Check sheet for the modelled part. Datum: model origin and axes. Units: mm. Face numbers are marked on the shaded views. Round coordinates to 2 decimals unless told otherwise and drop trailing zeros. Order: outer loops, then holes, each group sorted by start corner. A loop starts at its lowest first (then second) coordinate and runs counter-clockwise, first axis right, second up. Notation, with made-up numbers: (45.5, 57.5) -> (92.5, 57.5) arc R17 ccw to (92.5, 85.5) -> close; hole circle Ø7 at (87, 39.5). An arc over 180 degrees is marked (long way). Answer in a Markdown table with one row per item. Add a question column.
1. Sectioned sample at B-B, the plane y = -7.5. Record the boundary of the cut face in (x, z), then the cut area to 3 significant figures.
2. Sectioned sample at A-A, the plane z = 10.5. Record the boundary of the cut face in (x, y).
3. Sectioned sample at C-C, the plane x = 5.75. Record the boundary of the cut face in (y, z), then the cut area to 3 significant figures.
4. Draft check along X on the marked faces 1, 2, 3 and 4. Enter one of: +X half, -X half, draft (parallel to the pull), parting line (faces both ways), or undercut.
5. Material ranges on L1, parallel to Y at x = 0, z = 13; L2, parallel to X at y = 3.03, z = 10; L3, parallel to X at y = 2, z = 2, recorded low to high. Write a range as from..to.
```python
from build123d import *

# Parameters (mm, degrees)
SKETCH1_W             = 15
SKETCH1_H             = 20
BOSS_EXTRUDE1_DEPTH   = 17.5
CHAMFER1_SIZE         = 3
M6_TAPPED_HOLE1_D     = 5
M6_TAPPED_HOLE1_DEPTH = 15
M6_TAPPED_HOLE1_TIP   = 1.502151548


with BuildPart() as part:
    # Sketch1 → Boss-Extrude1 (new, symmetric)
    with BuildSketch(Plane.XY):
        Rectangle(SKETCH1_W, SKETCH1_H)
    extrude(amount=BOSS_EXTRUDE1_DEPTH, both=True)

    # Chamfer1
    chamfer1_edges = [part.edges().sort_by_distance(p)[0] for p in [
        (7.5, -10, 0),
        (-7.5, -10, 0),
    ]]
    chamfer(chamfer1_edges, length=CHAMFER1_SIZE)

    # M6 Tapped Hole1
    with Locations(Plane.XY.offset(17.5)):
        with Locations((0, 3.03)):
            Hole(M6_TAPPED_HOLE1_D / 2, depth=M6_TAPPED_HOLE1_DEPTH)
            with Locations((0, 0, -(M6_TAPPED_HOLE1_DEPTH + M6_TAPPED_HOLE1_TIP / 2))):  # 118° drill point
                Cone(0, M6_TAPPED_HOLE1_D / 2, M6_TAPPED_HOLE1_TIP, mode=Mode.SUBTRACT)


solid = part.part
```
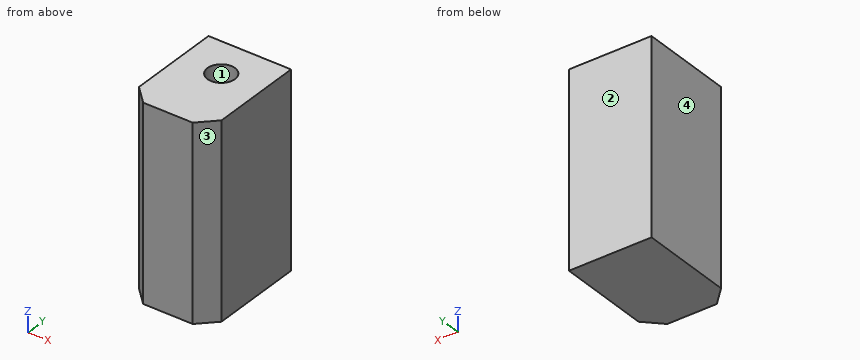
Answer key:
| question | item | result |
|---|---|---|
| 1 | outline | (-7, -17.5) -> (7, -17.5) -> (7, 17.5) -> (-7, 17.5) -> close |
| 1 | area | 490 mm² |
| 2 | outline | (-7.5, -7) -> (-4.5, -10) -> (4.5, -10) -> (7.5, -7) -> (7.5, 10) -> (-7.5, 10) -> close; hole circle Ø5 at (0, 3.03) |
| 3 | outline | (-8.75, -17.5) -> (10, -17.5) -> (10, 17.5) -> (-8.75, 17.5) -> close |
| 3 | area | 656 mm² |
| 4 | face 1 | undercut |
| 4 | face 2 | draft |
| 4 | face 3 | +X half |
| 4 | face 4 | -X half |
| 5 | L1 | y = -10..0.53, 5.53..10 |
| 5 | L2 | x = -7.5..-2.5, 2.5..7.5 |
| 5 | L3 | x = -7.5..-1.31, 1.31..7.5 |
